```python
from build123d import *

# Parameters (mm, degrees)
SCALE_1_SCALE = 1.875


with BuildPart() as part:
    # Sketch1 → Revolve1 (revolve)
    with BuildSketch(Plane.XY, mode=Mode.PRIVATE) as revolve1_sk:
        with BuildLine():
            Line((4, -40), (4, -111))
            Line((4, -111), (2, -112))
            Line((2, -112), (0, -112))
            Line((0, -112), (0, 2))
            Line((0, 2), (14, 2))
            Line((14, 2), (16, 0))
            Line((16, 0), (16, -6))
            Line((16, -6), (14, -8))
            ThreePointArc((14, -8), (9.860217357, -13.169110669), (13, -19))
            Line((13, -19), (13, -25))
            Line((13, -25), (6.5, -25))
            Line((6.5, -25), (6.5, -28))
            Line((6.5, -28), (10, -28))
            Line((10, -28), (10, -39))
            Line((10, -39), (9, -40))
            Line((9, -40), (4, -40))
        make_face()
    revolve(revolve1_sk.sketch.rotate(Axis((0, 2, 0), (0, -1, 0)), 90), axis=Axis((0, 2, 0), (0, -1, 0)))


with BuildPart() as part_1:
    # Scale 1: scaled about (0, -24.610702711, 0)
    add(part.part.scale(SCALE_1_SCALE).moved(Location((0, 21.534364872, 0))))


solid = part_1.part
```
For this review, take the finished solid that the model builds, in its own axes (mm). A direction names the side the tool comes from. Give positions to 0.01 mm unless a question says otherwise; leave off trailing zeros. Write each loop counter-clockwise with the first axis right and the second up, starting at its lowest first coordinate (ties: lowest second). Pieces come first, ordered by that corner, then holes. Notation, with made-up numbers: M 55.25,27 L 60.25,27 A17 ccw 60.25,55 Z; hole C 14,6 d6. An arc over 180 degrees is marked long. Answer as a JSON object with one key per item and string values. Group by question number.
Item 1: For pin 1 Ø5 at (y, z) = (-77.5, -3) entering from +X; pin 2 Ø10 at (y, z) = (-105, 13) entering from +X; pin 3 Ø8 at (x, z) = (-12.5, 23.5) entering from -Y; pin 4 Ø2 at (y, z) = (-33.5, 6) entering from +X, all flat-tipped, find the tip position at first contact; note any pin that passes through.
Item 2: For probe 1 along Y at (x, z) = (5.5, -8.5); probe 2 along Y at (x, z) = (-4, -23); probe 3 along Z at (x, y) = (-4, -75.5), list the stretches that pass through material, from the lowest coordinate up. Write a range as [from, to].
Item 3: Consider section D-D on y = -19.5. Write out the cut boundary in (x, z) (3 decimals).
Item 4: Tool access review of faces 5 (the flat face through (0, 25.284, 0)), 6 (the cylindrical face through (7.42, -28.19, -9.67)), 7 (the flat face through (7, -53.466, 4)): name each direction out of +Z, -Z, +X, -X, +Y, -Y from which nothing blocks a thin tool from reaching the whole face with its end or side.
Item 5: Consider section C-C on y = -101. Write out the cut boundary in (x, z), plus the area to 3 significant figures.
Item 6: Draft analysis for pull direction Y (two halves, no side actions). For faces 1 (the conical face through (-1.181, -188.375, 3.751)), 2 (the conical face through (-8, 25, 25.3)), 3 (the cylindrical face through (-25.296, 15.831, 16.128)), 4 (the flat face through (12, -30.966, -4)), state which applies: +Y half, -Y half, draft (parallel to the pull), parting line (faces both ways), or undercut.
Check result:
{
 "1": {"pin 1": "stops at x = 7.48", "pin 2": "passes through", "pin 3": "stops at y = -25.34", "pin 4": "stops at x = 18.07"},
 "2": {"probe 1": "y = [-53.47, 25.28]", "probe 2": "y = [-25.34, -13.47], [5.11, 25.28]", "probe 3": "z = [-6.34, 6.34]"},
 "3": {"outline": "C 0,0 d48.75"},
 "4": {"face 5": "+Z, -Z, +X, -X, +Y", "face 6": "none", "face 7": "-Y"},
 "5": {"outline": "C 0,0 d15", "area": "177 mm^2"},
 "6": {"face 1": "-Y half", "face 2": "+Y half", "face 3": "draft", "face 4": "undercut"}
}
